Source: CAD feature listing. Evaluate the final solid. Frame: model axes, mm. Face numbers are marked on the shaded views. Coordinates: 2 decimals unless noted, no trailing zeros. Order: outer loops, then holes, each group sorted by start corner. A loop starts at its lowest first (then second) coordinate and runs counter-clockwise, first axis right, second up.
Item 1: Mould query, pull axis X, two halves, no side actions, for the marked faces 1, 2 and 3. Classes: released by +X, released by -X, zero draft, split by the parting line, or undercut.
Item 2: Section D-D on z = 10. State how many separate pieces and enclosed holes the cut face has, then the cut area to 3 significant figures.
Item 3: Ray query, line 1 (X direction, y = 36, z = 7.5); line 2 (X direction, y = 33.5, z = 6); line 3 (Y direction, x = 34, z = 7.5). Return the intervals inside material, ascending.
Item 4: Section C-C on y = 50.5. Return the cut outline in (x, z), then the cut area to 3 significant figures.
Item 5: Contact query for flat-ended pins moving along their axis: P1, Ø1.5, axis at x = -36, z = 8, coming from the +Y side; P2, Ø1, axis at x = 26, y = -22, coming from the +Z side; P3, Ø1, axis at x = 39, z = 2.5, coming from the +Y side. Output: stop coordinate, or through.
Item 6: Section B-B on x = 24. Return the cut outline in (y, z).
Item 7: Section A-A on y = 0. Return the cut outline in (x, z), then the cut area to 3 significant figures.
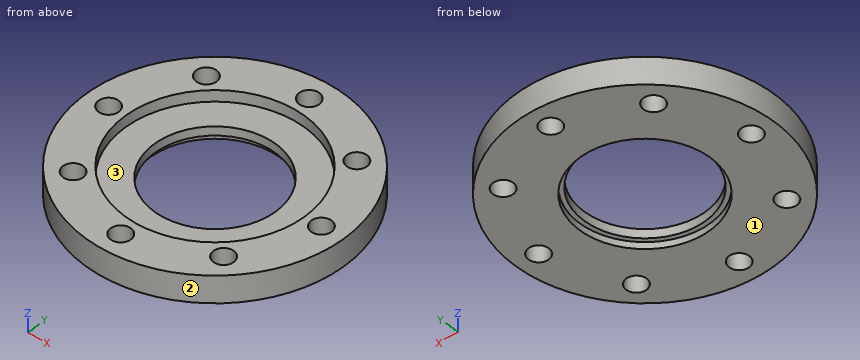
from build123d import *

# Parameters (mm, degrees)
SKETCH_1_R          = 57.5
EXTRUDE_1_DEPTH     = 12
SKETCH_2_R          = 40
CUT_EXTRUDE_1_DEPTH = 5
SKETCH_3_R          = 27
CUT_EXTRUDE_2_DEPTH = 13
SKETCH_4_R          = 29
CUT_EXTRUDE_3_DEPTH = 3
SKETCH_5_R          = 4.5
CUT_EXTRUDE_4_DEPTH = 50


with BuildPart() as part:
    # 草图1 → 凸台-拉伸1 (new body)
    with BuildSketch(Plane.XY):
        Circle(SKETCH_1_R)
    extrude(amount=EXTRUDE_1_DEPTH)

    # 草图2 → 切除-拉伸1 (cut)
    with BuildSketch(Plane.XY.offset(12)):
        Circle(SKETCH_2_R)
    extrude(amount=-CUT_EXTRUDE_1_DEPTH, mode=Mode.SUBTRACT)

    # 草图3 → 切除-拉伸2 (cut)
    with BuildSketch(Plane.XY.offset(7)):
        Circle(SKETCH_3_R)
    extrude(amount=-CUT_EXTRUDE_2_DEPTH, mode=Mode.SUBTRACT)

    # 草图4 → 切除-拉伸3 (cut)
    with BuildSketch(Plane(origin=(0, 0, 0), x_dir=(-1, 0, 0), z_dir=(0, 0, -1))):
        Circle(SKETCH_4_R)
    extrude(amount=-CUT_EXTRUDE_3_DEPTH, mode=Mode.SUBTRACT)

    # 草图5 → 切除-拉伸4 (cut)
    with BuildSketch(Plane.XY.offset(12)):
        with Locations((0, 47.5)):
            Circle(SKETCH_5_R)
        with Locations((33.587572106, 33.587572106)):
            Circle(SKETCH_5_R)
        with Locations((47.5, 0)):
            Circle(SKETCH_5_R)
        with Locations((33.587572106, -33.587572106)):
            Circle(SKETCH_5_R)
        with Locations((0, -47.5)):
            Circle(SKETCH_5_R)
        with Locations((-33.587572106, -33.587572106)):
            Circle(SKETCH_5_R)
        with Locations((-47.5, 0)):
            Circle(SKETCH_5_R)
        with Locations((-33.587572106, 33.587572106)):
            Circle(SKETCH_5_R)
    extrude(amount=-CUT_EXTRUDE_4_DEPTH, mode=Mode.SUBTRACT)


solid = part.part
Answer list:
1. face 1: zero draft
1. face 2: split by the parting line
1. face 3: undercut
2. separate pieces: 1
2. enclosed holes: 9
2. area: 4,850 mm2
3. line 1: x = -44.84 to -37.39, -29.79 to -17.44, 17.44 to 29.79, 37.39 to 44.84
3. line 2: x = -46.73 to -38.09, -29.09 to 29.09, 38.09 to 46.73
3. line 3: y = -46.37 to -38.07, -29.11 to -21.07, 21.07 to 29.11, 38.07 to 46.37
4. outline: (-27.5, 0) - (-3.35, 0) - (-3.35, 12) - (-27.5, 12) - close; (3.35, 0) - (27.5, 0) - (27.5, 12) - (3.35, 12) - close
4. area: 579 mm2
5. P1: stops at y = 45.43
5. P2: stops at z = 7
5. P3: stops at y = 42.71
6. outline: (-52.25, 0) - (-16.28, 0) - (-16.28, 3) - (-12.37, 3) - (-12.37, 7) - (-32, 7) - (-32, 12) - (-52.25, 12) - close; (12.37, 3) - (16.28, 3) - (16.28, 0) - (52.25, 0) - (52.25, 12) - (32, 12) - (32, 7) - (12.37, 7) - close
7. outline: (-57.5, 0) - (-52, 0) - (-52, 12) - (-57.5, 12) - close; (-43, 0) - (-29, 0) - (-29, 3) - (-27, 3) - (-27, 7) - (-40, 7) - (-40, 12) - (-43, 12) - close; (27, 3) - (29, 3) - (29, 0) - (43, 0) - (43, 12) - (40, 12) - (40, 7) - (27, 7) - close; (52, 0) - (57.5, 0) - (57.5, 12) - (52, 12) - close
7. area: 374 mm2
